from build123d import *

# Parameters (mm, degrees)
SKETCH1_W           = 7
SKETCH1_H           = 8
BOSS_EXTRUDE1_DEPTH = 10
SKETCH2_W           = 7
SKETCH2_H           = 2
BOSS_EXTRUDE2_DEPTH = 8
SKETCH3_R           = 1
BOSS_EXTRUDE3_DEPTH = 5
FILLET1_R           = 0.5
SKETCH4_R           = 1.490192279
BOSS_EXTRUDE4_DEPTH = 1
SKETCH5_R           = 1.426715447
BOSS_EXTRUDE5_DEPTH = 0.5
FILLET3_R           = 0.5
FILLET4_R           = 1
SKETCH6_R           = 1.75
CUT_EXTRUDE1_DEPTH  = 20.293781382


with BuildPart() as part:
    # Sketch1 → Boss-Extrude1 (new body)
    with BuildSketch(Plane.XY):
        Rectangle(SKETCH1_W, SKETCH1_H)
    extrude(amount=BOSS_EXTRUDE1_DEPTH)

    # Sketch2 → Boss-Extrude2 (add)
    with BuildSketch(Plane.XY.offset(10)):
        with Locations((0, -3)):
            Rectangle(SKETCH2_W, SKETCH2_H)
    extrude(amount=BOSS_EXTRUDE2_DEPTH)

    # Sketch3 → Boss-Extrude3 (add)
    with BuildSketch(Plane(origin=(0, 0, 0), x_dir=(-1, 0, 0), z_dir=(0, 0, -1))):
        Circle(SKETCH3_R)
    extrude(amount=BOSS_EXTRUDE3_DEPTH)

    # Fillet1
    fillet1_edges = [part.edges().sort_by_distance(p)[0] for p in [
        (1, 0, -5),
    ]]
    fillet(fillet1_edges, radius=FILLET1_R)

    # Sketch4 → Boss-Extrude4 (add)
    with BuildSketch(Plane(origin=(0, 0, 0), x_dir=(-1, 0, 0), z_dir=(0, 0, -1))):
        with Locations(Location((0, 0, 0), (0, 0, 180))):
            Circle(SKETCH4_R)
    extrude(amount=BOSS_EXTRUDE4_DEPTH)

    # Sketch5 → Boss-Extrude5 (add)
    with BuildSketch(Plane.XY.offset(10)):
        Circle(SKETCH5_R)
    extrude(amount=BOSS_EXTRUDE5_DEPTH)

    # Fillet3
    fillet3_edges = [part.edges().sort_by_distance(p)[0] for p in [
        (-3.5, 4, 5),
        (3.5, 4, 5),
    ]]
    fillet(fillet3_edges, radius=FILLET3_R)

    # Fillet4
    fillet4_edges = [part.edges().sort_by_distance(p)[0] for p in [
        (3.5, -3, 18),
        (-3.5, -3, 18),
    ]]
    fillet(fillet4_edges, radius=FILLET4_R)

    # Sketch6 → Cut-Extrude1 (cut, through all)
    with BuildSketch(Plane(origin=(0, -2, 0), x_dir=(1, 0, 0), z_dir=(0, 1, 0))):
        with Locations(Location((0, -14.5, 0), (0, 0, 270))):
            Circle(SKETCH6_R)
    extrude(amount=-CUT_EXTRUDE1_DEPTH, mode=Mode.SUBTRACT)


solid = part.part
Work out the finished part from the listing and answer in its coordinate system (mm). A direction names the side the tool comes from. Round coordinates to 2 decimals unless told otherwise and drop trailing zeros. Loops run counter-clockwise (first coordinate to the right, second up) from the corner with the lowest first, then second, coordinate; pieces in that order, holes last. Notation, with made-up numbers: (-38, 39) - (-13, 39) arc R16 ccw to (-13, 68) - close; hole circle Ø7 at (7.25, 6). An arc over 180 degrees is marked (long way). Use one line per item in the form item = value. Start each with the question number.
(1) Find section C-C on z = -3. Determine the outline of the cut face in (x, y), and give its area (3 significant figures).
(2) Determine the mould class of faces 3 (the face through (0.526, -2.986, 16.169)), 4 (the face through (1.36, 0.43, 10.25)), 5 (the face through (0, 0, 10.5)) for opening direction X: +X half, -X half, draft (parallel to the pull), parting line (faces both ways), or undercut.
(3) Find section B-B on y = 2. Determine the outline of the cut face in (x, z).
(4) Consider line 1 (X direction, y = -3.2, z = 14.5); line 2 (Y direction, x = 1.25, z = 12.5); line 3 (Z direction, x = 0.5, y = -3). Determine where each line is inside the solid, lowest interval first.
(5) Find section A-A on z = 14.75. Determine the outline of the cut face in (x, y).
(6) Which of the six approach directions +Z, -Z, +X, -X, +Y, -Y give full straight-line access (tool end or side, diameter ignored) to faces 1 (the face through (-3.215, -2.986, 17.699)), 2 (the face through (0, -1, -3))?
(7) Flat-ended cylindrical pins translate along their axes: P1, Ø2, axis at x = -1.5, y = -0.5, coming from the -Z side; P2, Ø1.8, axis at x = 1.5, y = 2, coming from the +Z side; P3, Ø3.5, axis at x = -1, z = 15.5, coming from the +Y side. Find the tip coordinate at first contact, or state that the pin passes through.
Answer list:
q1.outline = circle Ø2 at (0, 0)
q1.area = 3.14 mm^2
q2.face_3 = undercut
q2.face_4 = parting line
q2.face_5 = draft
q3.outline = (-3.5, 0) - (3.5, 0) - (3.5, 10) - (-3.5, 10) - close
q4.line_1 = -3.5 to -1.75, 1.75 to 3.5
q4.line_2 = -4 to -2
q4.line_3 = 0 to 12.82, 16.18 to 18
q5.outline = (-3.5, -4) - (-1.73, -4) - (-1.73, -2) - (-3.5, -2) - close; (1.73, -4) - (3.5, -4) - (3.5, -2) - (1.73, -2) - close
q6.face_1 = +Z, -X, +Y, -Y
q6.face_2 = -Z
q7.P1 = -4.99
q7.P2 = 10
q7.P3 = -2
